Source: CAD feature listing. Evaluate the final solid. Frame: model axes, mm. A direction names the side the tool comes from. Round coordinates to 2 decimals unless told otherwise and drop trailing zeros. Order: outer loops, then holes, each group sorted by start corner. A loop starts at its lowest first (then second) coordinate and runs counter-clockwise, first axis right, second up. Notation, with made-up numbers: M 23.5,-18 L 60.5,-18 A26 cw 60.5,0 Z; hole C 32,-17 d6. An arc over 180 degrees is marked long. Answer in a Markdown table with one row per item. Add a question column.
```python
from build123d import *

# Parameters (mm, degrees)
SKETCH_1_R                = 30
EXTRUDE_1_DEPTH           = 10
M20X1_5_1_D               = 18.5
HOLE_WIZARD_1_D           = 4.5
HOLE_WIZARD_1_CBORE_D     = 8
HOLE_WIZARD_1_CBORE_DEPTH = 4.6
CHAMFER_1_SIZE            = 0.5


with BuildPart() as part:
    # 草图1 → 凸台-拉伸1 (new body)
    with BuildSketch(Plane(origin=(0, 0, 0), x_dir=(1, 0, 0), z_dir=(0, 1, 0))):
        with Locations(Location((0, 0, 0), (0, 0, 270))):
            Circle(SKETCH_1_R)
    extrude(amount=EXTRUDE_1_DEPTH)

    # M20x1.5 螺纹孔1 (through all)
    with Locations(Plane(origin=(0, 10, 0), x_dir=(1, 0, 0), z_dir=(0, 1, 0))):
        with Locations((0, 0)):
            Hole(M20X1_5_1_D / 2)

    # 打孔尺寸(%根据)内六角圆柱头螺钉的类型1 (through all)
    with Locations(Plane(origin=(0, 10, 0), x_dir=(1, 0, 0), z_dir=(0, 1, 0))):
        with Locations((0, 25), (25, 0), (0, -25), (-25, 0)):
            CounterBoreHole(HOLE_WIZARD_1_D / 2, HOLE_WIZARD_1_CBORE_D / 2, HOLE_WIZARD_1_CBORE_DEPTH)

    # 倒角1
    chamfer_1_edges = [part.edges().sort_by_distance(p)[0] for p in [
        (0, 0, -30),
        (0, 10, -30),
        (9.25, 10, 0),
        (9.25, 0, 0),
    ]]
    chamfer(chamfer_1_edges, length=CHAMFER_1_SIZE)


solid = part.part
```
(1) Cut plane A-A (y = 2.5). Return loops of the section in (x, z), and give its area (3 significant figures).
(2) Cut plane B-B (z = 0). Count the separate pieces of the cut face and the enclosed holes in it, and give its area (3 significant figures).
(3) Pin query (flat end, axial travel): pin 1 (2 mm diameter, centred on y = 3, z = 9.5, fed in from -X); pin 2 (4 mm diameter, centred on x = 1.5, z = 26, fed in from +Y); pin 3 (2 mm diameter, centred on x = 6.5, y = 4.5, fed in from -Z). Return the tip coordinate at first contact, or that it passes through.
(4) Cut plane D-D (y = 6.25). Return loops of the section in (x, z).
(5) Access query for faces 1 (the face through (-28.2, 7.7, 2.4)), 2 (the face through (-27.146, 2.662, -0.676)). Directions: +Z, -Z, +X, -X, +Y, -Y. A direction counts if a zero-diameter tool reaches every point of the face in a straight line with its end or side. Return the directions, or none.
(6) Line query: line 1 (X direction, y = 2.5, z = -2); line 2 (Y direction, x = 27.5, z = -3); line 3 (Z direction, x = -25, y = 2.3). Output: solid intervals per line, ascending. Write a range as from..to.
(7) Draft query along Z for faces 3 (the face through (0, 10, 13)), 4 (the face through (2.01, 4.94, 9.03)), 5 (the face through (1.32, 4.94, -29.97)). Return one class per face: +Z half, -Z half, draft (parallel to the pull), parting line (faces both ways), or undercut.
Answer list:
| question | item | result |
|---|---|---|
| 1 | outline | C 0,0 d60; hole C -25,0 d4.5; hole C 0,0 d18.5; hole C 0,-25 d4.5; hole C 0,25 d4.5; hole C 25,0 d4.5 |
| 1 | area | 2,500 mm² |
| 2 | separate pieces | 4 |
| 2 | enclosed holes | 0 |
| 2 | area | 292 mm² |
| 3 | pin 1 | x = -28.77 |
| 3 | pin 2 | y = 5.4 |
| 3 | pin 3 | z = -29.49 |
| 4 | outline | C 0,0 d60; hole C -25,0 d8; hole C 0,0 d18.5; hole C 0,-25 d8; hole C 0,25 d8; hole C 25,0 d8 |
| 5 | face 1 | +Y |
| 5 | face 2 | +Y, -Y |
| 6 | line 1 | -29.93..-26.03, -23.97..-9.03, 9.03..23.97, 26.03..29.93 |
| 6 | line 2 | 0..5.4 |
| 6 | line 3 | -16.58..-2.25, 2.25..16.58 |
| 7 | face 3 | draft |
| 7 | face 4 | undercut |
| 7 | face 5 | parting line |
